The listing builds one solid part. Answer for the finished solid, in the listing's coordinates (mm). A direction names the side the tool comes from. Give positions to 0.01 mm unless a question says otherwise; leave off trailing zeros. Order: outer loops, then holes, each group sorted by start corner. A loop starts at its lowest first (then second) coordinate and runs counter-clockwise, first axis right, second up. Notation, with made-up numbers: (68, 49.25) -> (89, 49.25) arc R27 cw to (89, 85.25) -> close; hole circle Ø11 at (48, -34). An arc over 180 degrees is marked (long way). Answer as a JSON object with one key per item and string values. Group by question number.
```python
from build123d import *

# Parameters (mm, degrees)
SKETCH1_R               = 40
BOSS_EXTRUDE1_DEPTH     = 18
CHAMFER2_SIZE           = 0.5
CUT_EXTRUDE1_DEPTH      = 60.363288319
CUT_EXTRUDE1_DEPTH_BACK = 60.363288319
SKETCH2_R               = 2.25
CUT_EXTRUDE2_DEPTH      = 4
CUT_EXTRUDE3_DEPTH      = 60.363288319
SKETCH5_R               = 9
CUT_EXTRUDE4_DEPTH      = 58.967380496
CUT_EXTRUDE5_DEPTH      = 16
SKETCH7_R               = 18.5
SKETCH7_R_2             = 14.5
CUT_EXTRUDE6_DEPTH      = 3
CHAMFER1_SIZE           = 0.5


with BuildPart() as part:
    # Sketch1 → Boss-Extrude1 (new body)
    with BuildSketch(Plane(origin=(0, 0, 0), x_dir=(1, 0, 0), z_dir=(0, 1, 0))):
        with Locations(Location((0, 0, 0), (0, 0, 270))):
            Circle(SKETCH1_R)
    extrude(amount=BOSS_EXTRUDE1_DEPTH)

    # Chamfer2
    chamfer2_edges = [part.edges().sort_by_distance(p)[0] for p in [
        (0, 0, -40),
        (0, 18, -40),
    ]]
    chamfer(chamfer2_edges, length=CHAMFER2_SIZE)

    # Sketch2 → Cut-Extrude1 (cut, two sides: drawn at the far end of the back side and taken through both)
    with BuildSketch(Plane(origin=(0, 18, 0), x_dir=(1, 0, 0), z_dir=(0, 1, 0)).offset(-CUT_EXTRUDE1_DEPTH_BACK)):
        with Locations(Location((36, 0, 0), (0, 0, 270))):
            Circle(SKETCH2_R)
        with Locations(Location((-36, 0, 0), (0, 0, 270))):
            Circle(SKETCH2_R)
    extrude(amount=CUT_EXTRUDE1_DEPTH + CUT_EXTRUDE1_DEPTH_BACK, mode=Mode.SUBTRACT)

    # Sketch3 → Cut-Extrude2 (cut)
    with BuildSketch(Plane(origin=(0, 18, 0), x_dir=(1, 0, 0), z_dir=(0, 1, 0))):
        with BuildLine():
            ThreePointArc((-25.162362394, 9.790583167), (-27, 0), (-25.162362394, -9.790583167))
            ThreePointArc((-25.162362394, -9.790583167), (-28.751993608, -13.771496887), (-29.807321036, -8.516079652))
            ThreePointArc((-29.807321036, -8.516079652), (-31, 0), (-29.807321036, 8.516079652))
            ThreePointArc((-29.807321036, 8.516079652), (-28.751993608, 13.771496887), (-25.162362394, 9.790583167))
        make_face()
        with BuildLine():
            ThreePointArc((25.162362394, -9.790583167), (28.751993608, -13.771496887), (29.807321036, -8.516079652))
            ThreePointArc((29.807321036, -8.516079652), (31, 0), (29.807321036, 8.516079652))
            ThreePointArc((29.807321036, 8.516079652), (28.751993608, 13.771496887), (25.162362394, 9.790583167))
            ThreePointArc((25.162362394, 9.790583167), (27, 0), (25.162362394, -9.790583167))
        make_face()
    extrude(amount=-CUT_EXTRUDE2_DEPTH, mode=Mode.SUBTRACT)

    # Sketch4 → Cut-Extrude3 (cut, through all)
    with BuildSketch(Plane(origin=(0, 18, 0), x_dir=(1, 0, 0), z_dir=(0, 1, 0))):
        with BuildLine():
            Line((-12.797765369, 37.8974564), (-9.02567097, 29.620350674))
            ThreePointArc((-9.02567097, 29.620350674), (-7.657078917, 28.191064594), (-5.696188381, 27.92496084))
            ThreePointArc((-5.696188381, 27.92496084), (0, 28.5), (5.696188381, 27.92496084))
            ThreePointArc((5.696188381, 27.92496084), (7.657078917, 28.191064594), (9.02567097, 29.620350674))
            Line((9.02567097, 29.620350674), (12.797765369, 37.8974564))
            ThreePointArc((12.797765369, 37.8974564), (0, 40), (-12.797765369, 37.8974564))
        make_face()
        with BuildLine():
            Line((12.797765369, -37.8974564), (9.02567097, -29.620350674))
            ThreePointArc((9.02567097, -29.620350674), (7.657078917, -28.191064594), (5.696188381, -27.92496084))
            ThreePointArc((5.696188381, -27.92496084), (0, -28.5), (-5.696188381, -27.92496084))
            ThreePointArc((-5.696188381, -27.92496084), (-7.657078917, -28.191064594), (-9.02567097, -29.620350674))
            Line((-9.02567097, -29.620350674), (-12.797765369, -37.8974564))
            ThreePointArc((-12.797765369, -37.8974564), (0, -40), (12.797765369, -37.8974564))
        make_face()
    extrude(amount=-CUT_EXTRUDE3_DEPTH, mode=Mode.SUBTRACT)

    # Sketch5 → Cut-Extrude4 (cut, through all)
    with BuildSketch(Plane(origin=(0, 0, 0), x_dir=(-1, 0, 0), z_dir=(0, -1, 0))):
        with Locations(Location((0, 0, 0), (0, 0, 90))):
            Circle(SKETCH5_R)
    extrude(amount=-CUT_EXTRUDE4_DEPTH, mode=Mode.SUBTRACT)

    # Sketch6 → Cut-Extrude5 (cut)
    with BuildSketch(Plane(origin=(0, 0, 0), x_dir=(-1, 0, 0), z_dir=(0, -1, 0))):
        with BuildLine():
            Line((17.529506166, -35.95436571), (11.275186187, -25.12156574))
            ThreePointArc((11.275186187, -25.12156574), (9.750918079, -23.820327414), (7.747419621, -23.769255125))
            ThreePointArc((7.747419621, -23.769255125), (0, -25), (-7.747419621, -23.769255125))
            ThreePointArc((-7.747419621, -23.769255125), (-9.750918079, -23.820327414), (-11.275186187, -25.12156574))
            Line((-11.275186187, -25.12156574), (-17.529506166, -35.95436571))
            ThreePointArc((-17.529506166, -35.95436571), (0, -40), (17.529506166, -35.95436571))
        make_face()
        with BuildLine():
            Line((-17.529506166, 35.95436571), (-11.275186187, 25.12156574))
            ThreePointArc((-11.275186187, 25.12156574), (-9.750918079, 23.820327414), (-7.747419621, 23.769255125))
            ThreePointArc((-7.747419621, 23.769255125), (0, 25), (7.747419621, 23.769255125))
            ThreePointArc((7.747419621, 23.769255125), (9.750918079, 23.820327414), (11.275186187, 25.12156574))
            Line((11.275186187, 25.12156574), (17.529506166, 35.95436571))
            ThreePointArc((17.529506166, 35.95436571), (0, 40), (-17.529506166, 35.95436571))
        make_face()
    extrude(amount=-CUT_EXTRUDE5_DEPTH, mode=Mode.SUBTRACT)

    # Sketch7 → Cut-Extrude6 (cut)
    with BuildSketch(Plane(origin=(0, 18, 0), x_dir=(1, 0, 0), z_dir=(0, 1, 0))):
        with Locations(Location((0, 0, 0), (0, 0, 270))):
            Circle(SKETCH7_R)
        with Locations(Location((0, 0, 0), (0, 0, 270))):
            Circle(SKETCH7_R_2, mode=Mode.SUBTRACT)
    extrude(amount=-CUT_EXTRUDE6_DEPTH, mode=Mode.SUBTRACT)

    # Chamfer1
    chamfer1_edges = [part.edges().sort_by_distance(p)[0] for p in [
        (0, 18, 9),
        (0, 0, 9),
    ]]
    chamfer(chamfer1_edges, length=CHAMFER1_SIZE)


solid = part.part
```
(1) A cutting plane is placed at B-B (y = 8.5). Determine the outline of the cut face in (x, z).
(2) Flat-ended cylindrical pins translate along their axes: pin 1 Ø11.5 at (x, z) = (-7, 30.5) entering from -Y; pin 2 Ø4 at (x, y) = (21, 4.5) entering from -Z; pin 3 Ø10 at (x, y) = (19, 11) entering from +Z. Find the tip coordinate at first contact, or state that the pin passes through.
(3) Find the intervals of material crossed by line 1 along X through (y, z) = (16.75, -6); line 2 along Y through (x, z) = (-17, 6); line 3 along Y through (x, z) = (28.5, -3.5), in increasing order. Write a range as [from, to].
(4) Which of the six approach directions +Z, -Z, +X, -X, +Y, -Y give full straight-line access (tool end or side, diameter ignored) to faces 4 (the cylindrical face through (-7.682, 17.014, -28.204)), 5 (the cylindrical face through (28.841, 16.028, -13.746)), 6 (the cylindrical face through (0, 8, 25))?
(5) A cutting plane is placed at A-A (x = 0). Determine the outline of the cut face in (y, z).
(6) For a pull along Z with two mould halves and no side action, classify faces 1 (the conical face through (-39.629, 17.865, -0.692)), 2 (the cylindrical face through (-31, 16, 0)), 3 (the cylindrical face through (7.682, 17.014, 28.204)) as +Z half, -Z half, draft (parallel to the pull), parting line (faces both ways), or undercut.
(7) A cutting plane is placed at C-C (z = 0). State how many separate pieces and enclosed holes the cut face has, and give its area (3 significant figures).
Check sheet entries:
{
 "1": {"outline": "(-17.53, -35.95) -> (-11.28, -25.12) arc R3 cw to (-7.75, -23.77) arc R25 ccw to (7.75, -23.77) arc R3 cw to (11.28, -25.12) -> (17.53, -35.95) arc R40 ccw to (17.53, 35.95) -> (11.28, 25.12) arc R3 cw to (7.75, 23.77) arc R25 ccw to (-7.75, 23.77) arc R3 cw to (-11.28, 25.12) -> (-17.53, 35.95) arc R40 ccw to start; hole circle Ø4.5 at (-36, 0); hole circle Ø18 at (0, 0); hole circle Ø4.5 at (36, 0)"},
 "2": {"pin 1": "stops at y = 16", "pin 2": "stops at z = -35.2", "pin 3": "stops at z = 35.95"},
 "3": {"line 1": "x = [-39.55, -30.41], [-26.32, -17.5], [-13.2, -6.71], [6.71, 13.2], [17.5, 26.32], [30.41, 39.55]", "line 2": "y = [0, 15]", "line 3": "y = [0, 14]"},
 "4": {"face 4": "-Z, +Y, -Y", "face 5": "+Y", "face 6": "+Z, -Y"},
 "5": {"outline": "(0, -25) -> (16, -25) -> (16, -28.5) -> (18, -28.5) -> (18, -18.5) -> (15, -18.5) -> (15, -14.5) -> (18, -14.5) -> (18, -9.5) -> (17.5, -9) -> (0.5, -9) -> (0, -9.5) -> close; (0, 9.5) -> (0.5, 9) -> (17.5, 9) -> (18, 9.5) -> (18, 14.5) -> (15, 14.5) -> (15, 18.5) -> (18, 18.5) -> (18, 28.5) -> (16, 28.5) -> (16, 25) -> (0, 25) -> close"},
 "6": {"face 1": "parting line", "face 2": "undercut", "face 3": "+Z half"},
 "7": {"separate pieces": "4", "enclosed holes": "0", "area": "897 mm2"}
}
